```python
from build123d import *


with BuildPart() as part:
    # 草图1 → 旋转1 (revolve)
    with BuildSketch(Plane.XY, mode=Mode.PRIVATE) as revolve_1_sk:
        Polygon((-94.709677419, 0), (-94.709677419, 12), (-42.709677419, 12), (-42.709677419, 15), (17.290322581, 15), (17.290322581, 20), (505.290322581, 20), (505.290322581, 15), (553.290322581, 15), (553.290322581, 12), (590.290322581, 12), (590.290322581, 0), align=None)
    revolve(revolve_1_sk.sketch.rotate(Axis((-124.903225806, 0, 0), (1, 0, 0)), 90), axis=Axis((-124.903225806, 0, 0), (1, 0, 0)))


solid = part.part
```
Build history of the part. All positions in model axes, mm. A direction names the side the tool comes from. Round coordinates to 2 decimals unless told otherwise and drop trailing zeros. Write each loop counter-clockwise with the first axis right and the second up, starting at its lowest first coordinate (ties: lowest second). Pieces come first, ordered by that corner, then holes.
1) 3-axis set-ups, long thin cutter, end or side, ignore diameter. For faces 1 (the cylindrical face through (-12.29, -12.65, 8.06)), 2 (the flat face through (505.29, -15, 3)), 3 (the flat face through (-94.71, 0, 0)): which of +Z, -Z, +X, -X, +Y, -Y reach the whole face in a straight line?
2) Pin check, flat tips, straight feed: pin 1 (1.5 mm diameter, centred on y = 14.5, z = -0.5, fed in from +X); pin 2 (6 mm diameter, centred on x = 158.5, z = -0.5, fed in from -Y); pin 3 (10 mm diameter, centred on y = -12, z = -14.5, fed in from -X); pin 4 (12 mm diameter, centred on x = 100, y = -4.5, fed in from +Z). Stop position of each tip, or through.
3) Band-saw the part on A-A, the plane z = 0. List the corners of the cut face in (x, y).
4) Drill centre lines: probe 1 along Z at (x, y) = (433.5, -1); probe 2 along X at (y, z) = (-18, -1); probe 3 along Y at (x, z) = (414.5, -2). Where is each one in solid material? Low to high.
5) Band-saw the part on C-C, the plane x = 3. List the corners of the cut face in (y, z).
Ans:
1. face 1: -X
1. face 2: +X
1. face 3: +Z, -Z, -X, +Y, -Y
2. pin 1: stops at x = 553.29
2. pin 2: stops at y = -20
2. pin 3: stops at x = -42.71
2. pin 4: stops at z = 20
3. outline: (-94.71, -12) - (-42.71, -12) - (-42.71, -15) - (17.29, -15) - (17.29, -20) - (505.29, -20) - (505.29, -15) - (553.29, -15) - (553.29, -12) - (590.29, -12) - (590.29, 12) - (553.29, 12) - (553.29, 15) - (505.29, 15) - (505.29, 20) - (17.29, 20) - (17.29, 15) - (-42.71, 15) - (-42.71, 12) - (-94.71, 12) - close
4. probe 1: z = -19.97 to 19.97
4. probe 2: x = 17.29 to 505.29
4. probe 3: y = -19.9 to 19.9
5. outline: circle Ø30 at (0, 0)
